```python
from build123d import *

# Parameters (mm, degrees)
SKETCH1_R           = 85
BOSS_EXTRUDE1_DEPTH = 215
CUT_EXTRUDE1_START  = 5
SKETCH2_R           = 110
SKETCH2_R_2         = 70
CUT_EXTRUDE1_DEPTH  = 140
FILLET1_R           = 2
SKETCH3_R           = 62.5
CUT_EXTRUDE2_DEPTH  = 25
CUT_EXTRUDE3_START  = -25
SKETCH4_R           = 62.5
CUT_EXTRUDE3_DEPTH  = 25
SKETCH5_R           = 52.5
CUT_EXTRUDE4_DEPTH  = 225.833271559


with BuildPart() as part:
    # Sketch1 → Boss-Extrude1 (new body)
    with BuildSketch(Plane(origin=(0, 0, 0), x_dir=(0, 0, -1), z_dir=(1, 0, 0))):
        Circle(SKETCH1_R)
    extrude(amount=BOSS_EXTRUDE1_DEPTH)

    # Sketch2 → Cut-Extrude1 (cut)
    with BuildSketch(Plane(origin=(172.5, 0, 0), x_dir=(0, 0, -1), z_dir=(1, 0, 0)).offset(CUT_EXTRUDE1_START)):
        Circle(SKETCH2_R)
        Circle(SKETCH2_R_2, mode=Mode.SUBTRACT)
    extrude(amount=-CUT_EXTRUDE1_DEPTH, mode=Mode.SUBTRACT)

    # Fillet1
    fillet1_edges = [part.edges().sort_by_distance(p)[0] for p in [
        (37.5, 0, 70),
        (177.5, 0, 70),
    ]]
    fillet(fillet1_edges, radius=FILLET1_R)

    # Sketch3 → Cut-Extrude2 (cut)
    with BuildSketch(Plane(origin=(215, 0, 0), x_dir=(0, 0, -1), z_dir=(1, 0, 0))):
        Circle(SKETCH3_R)
    extrude(amount=-CUT_EXTRUDE2_DEPTH, mode=Mode.SUBTRACT)

    # Sketch4 → Cut-Extrude3 (cut)
    with BuildSketch(Plane.ZY.offset(CUT_EXTRUDE3_START)):
        with Locations(Location((0, 0, 0), (0, 0, 180))):
            Circle(SKETCH4_R)
    extrude(amount=CUT_EXTRUDE3_DEPTH, mode=Mode.SUBTRACT)

    # Sketch5 → Cut-Extrude4 (cut, through all)
    with BuildSketch(Plane(origin=(190, 0, 0), x_dir=(0, 0, -1), z_dir=(1, 0, 0))):
        Circle(SKETCH5_R)
    extrude(amount=-CUT_EXTRUDE4_DEPTH, mode=Mode.SUBTRACT)


solid = part.part
```
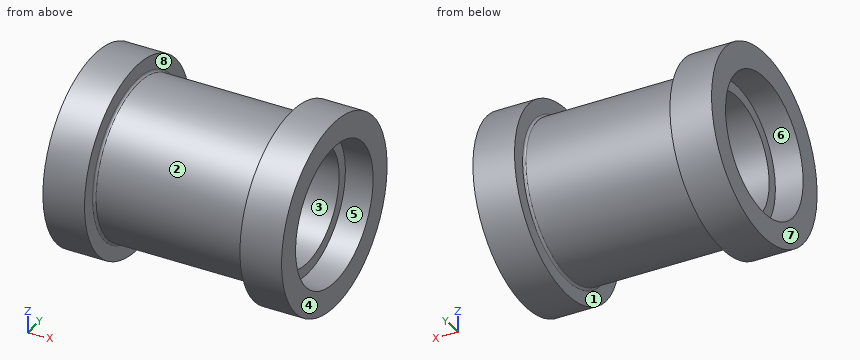
Build history of the part. All positions in model axes, mm. Face numbers are marked on the shaded views. A direction names the side the tool comes from. Give positions to 0.01 mm unless a question says otherwise; leave off trailing zeros. Order: outer loops, then holes, each group sorted by start corner. A loop starts at its lowest first (then second) coordinate and runs counter-clockwise, first axis right, second up. Notation, with made-up numbers: M -7.5,-33 L 38.5,-33 A29 cw 38.5,1 Z; hole C 54,31.5 d5. An arc over 180 degrees is marked long. Write item = value, one per line. Start each with the question number.
(1) Slice it at A-A on y = 0. Write the cut outline in (x, z), plus the area to 3 significant figures.
(2) Probe L1, parallel to X at y = 71, z = -24.5; L2, parallel to Y at x = 207.5, z = 0; L3, parallel to Y at x = 145, z = 0. List the from-to ranges inside material, lowest first. Write a range as [from, to].
(3) Which spindle directions (+Z, -Z, +X, -X, +Y, -Y) get a long thin tool onto all of the face, cutting with end or side? Do the marked faces 5, 6, 7 and 8. Say none if no direction does.
(4) Two-plate mould, pull along X, no slides. Class the marked faces 1, 2, 3 and 4: released by +X, released by -X, zero draft, split by the parting line, or undercut.
(5) Pin check, flat tips, straight feed: pin 1 Ø1.5 at (x, y) = (180.5, -40) entering from +Z; pin 2 Ø6 at (x, y) = (189, -62) entering from +Z; pin 3 Ø1.5 at (x, y) = (79, 15) entering from -Z. Stop position of each tip, or through.
(6) Slice it at C-C on x = 94.5. Write the cut outline in (y, z), plus the area to 3 significant figures.
Responses:
q1.outline = M 0,-85 L 37.5,-85 L 37.5,-72 A2 cw 39.5,-70 L 175.5,-70 A2 cw 177.5,-72 L 177.5,-85 L 215,-85 L 215,-62.5 L 190,-62.5 L 190,-52.5 L 25,-52.5 L 25,-62.5 L 0,-62.5 Z; M 0,62.5 L 25,62.5 L 25,52.5 L 190,52.5 L 190,62.5 L 215,62.5 L 215,85 L 177.5,85 L 177.5,72 A2 cw 175.5,70 L 39.5,70 A2 cw 37.5,72 L 37.5,85 L 0,85 Z
q1.area = 8,780 mm2
q2.L1 = [0, 37.5], [177.5, 215]
q2.L2 = [-85, -62.5], [62.5, 85]
q2.L3 = [-70, -52.5], [52.5, 70]
q3.face_5 = +X
q3.face_6 = -X
q3.face_7 = +Z, -Z, -X, +Y, -Y
q3.face_8 = none
q4.face_1 = undercut
q4.face_2 = undercut
q4.face_3 = zero draft
q4.face_4 = released by +X
q5.pin_1 = 75.4
q5.pin_2 = 61.19
q5.pin_3 = -68.53
q6.outline = C 0,0 d140; hole C 0,0 d105
q6.area = 6,730 mm2
